from build123d import *

# Parameters (mm, degrees)
SKETCH_1_W      = 100
SKETCH_1_H      = 12
EXTRUDE_1_DEPTH = 1.5


with BuildPart() as part:
    # 草图1 → 凸台-拉伸1 (new body)
    with BuildSketch(Plane.XY):
        Rectangle(SKETCH_1_W, SKETCH_1_H)
        with BuildLine():
            Line((-45, 4.5), (45, 4.5))
            ThreePointArc((45, 4.5), (46.5, 3), (45, 1.5))
            Line((45, 1.5), (-45, 1.5))
            ThreePointArc((-45, 1.5), (-46.5, 3), (-45, 4.5))
        make_face(mode=Mode.SUBTRACT)
        with BuildLine():
            Line((-45, -4.5), (45, -4.5))
            ThreePointArc((45, -4.5), (46.5, -3), (45, -1.5))
            Line((45, -1.5), (-45, -1.5))
            ThreePointArc((-45, -1.5), (-46.5, -3), (-45, -4.5))
        make_face(mode=Mode.SUBTRACT)
    extrude(amount=EXTRUDE_1_DEPTH)


solid = part.part
CAD build for the part. Positions are in the model's coordinates, mm. Give positions to 0.01 mm unless a question says otherwise; leave off trailing zeros. Write each loop counter-clockwise with the first axis right and the second up, starting at its lowest first coordinate (ties: lowest second). Pieces come first, ordered by that corner, then holes. Notation, with made-up numbers: (-17, -24) -> (6, -24) arc R35 ccw to (6, 10) -> close; hole circle Ø3 at (10, 64). An arc over 180 degrees is marked (long way). Return JSON: item names as keys, results as strings.
Item 1: Band-saw the part on B-B (x = 5.5). List the corners of the cut face in (y, z), then the cut area to 3 significant figures.
Answer below:
{"outline": "(-6, 0) -> (-4.5, 0) -> (-4.5, 1.5) -> (-6, 1.5) -> close; (-1.5, 0) -> (1.5, 0) -> (1.5, 1.5) -> (-1.5, 1.5) -> close; (4.5, 0) -> (6, 0) -> (6, 1.5) -> (4.5, 1.5) -> close", "area": "9.00 mm2"}
Item 2: Band-saw the part on C-C (z = 0.45). List the corners of the cut face in (x, y), then the cut area to 3 significant figures.
Answer below:
{"outline": "(-50, -6) -> (50, -6) -> (50, 6) -> (-50, 6) -> close; hole (-45, -4.5) -> (45, -4.5) arc R1.5 ccw to (45, -1.5) -> (-45, -1.5) arc R1.5 ccw to start; hole (-45, 1.5) -> (45, 1.5) arc R1.5 ccw to (45, 4.5) -> (-45, 4.5) arc R1.5 ccw to start", "area": "646 mm2"}
Item 3: Drill centre lines: probe 1 along Y at (x, z) = (-26.5, 0.4); probe 2 along X at (y, z) = (3, 0.4); probe 3 along X at (y, z) = (3.5, 0.5). Where is each one in solid material? Low to high.
Answer below:
{"probe 1": "y = -6 to -4.5, -1.5 to 1.5, 4.5 to 6", "probe 2": "x = -50 to -46.5, 46.5 to 50", "probe 3": "x = -50 to -46.41, 46.41 to 50"}
Item 4: Band-saw the part on A-A (y = -3). List the corners of the cut face in (x, z), then the cut area to 3 significant figures.
Answer below:
{"outline": "(-50, 0) -> (-46.5, 0) -> (-46.5, 1.5) -> (-50, 1.5) -> close; (46.5, 0) -> (50, 0) -> (50, 1.5) -> (46.5, 1.5) -> close", "area": "10.5 mm2"}
